Source: CAD feature listing. Evaluate the final solid. Frame: model axes, mm. Give positions to 0.01 mm unless a question says otherwise; leave off trailing zeros. Loops run counter-clockwise (first coordinate to the right, second up) from the corner with the lowest first, then second, coordinate; pieces in that order, holes last. Notation, with made-up numbers: (54, -30.75) -> (95, -30.75) arc R21 ccw to (95, 7.25) -> close; hole circle Ø7 at (-9.75, 35). An arc over 180 degrees is marked (long way). Put each result on its own line as item: value.
```python
from build123d import *

# Parameters (mm, degrees)
SKETCH_1_W         = 8
SKETCH_1_H         = 8
EXTRUDE_1_DEPTH    = 35
HOLE_WIZARD_M4_1_D = 3.3


with BuildPart() as part:
    # 草图1 → 凸台-拉伸1 (new body)
    with BuildSketch(Plane.XY):
        Rectangle(SKETCH_1_W, SKETCH_1_H)
    extrude(amount=EXTRUDE_1_DEPTH)

    # M4 螺纹孔1 (through all)
    with Locations(Plane(origin=(0, -4, 0), x_dir=(-1, 0, 0), z_dir=(0, -1, 0))):
        with Locations((0, -12), (0, -4)):
            Hole(HOLE_WIZARD_M4_1_D / 2)


solid = part.part
```
(1) Section A-A on y = 1.25. Return loops of the section in (x, z).
Calculated:
outline: (-4, 0) -> (4, 0) -> (4, 35) -> (-4, 35) -> close; hole circle Ø3.3 at (0, 4); hole circle Ø3.3 at (0, 12)
(2) Section C-C on z = 4. Return loops of the section in (x, y).
Calculated:
outline: (-4, -4) -> (-1.65, -4) -> (-1.65, 4) -> (-4, 4) -> close; (1.65, -4) -> (4, -4) -> (4, 4) -> (1.65, 4) -> close
(3) Draft query along X for faces 1 (the cylindrical face through (-0.4, 0.1, 13.6)), 2 (the flat face through (0, 4, 17)), 3 (the flat face through (4, 0, 17)). Return one class per face: released by +X, released by -X, zero draft, split by the parting line, or undercut.
Calculated:
face 1: undercut
face 2: zero draft
face 3: released by +X
(4) First-contact query: P1, Ø2.5, axis at x = 0, z = 4, coming from the +Y side. Flat tip, straight axial feed; report the tip coordinate or a pass-through.
Calculated:
P1: passes through
(5) Section B-B on x = 0. Return loops of the section in (y, z), then the cut area to 3 significant figures.
Calculated:
outline: (-4, 0) -> (4, 0) -> (4, 2.35) -> (-4, 2.35) -> close; (-4, 5.65) -> (4, 5.65) -> (4, 10.35) -> (-4, 10.35) -> close; (-4, 13.65) -> (4, 13.65) -> (4, 35) -> (-4, 35) -> close
area: 227 mm²
(6) Line query: probe 1 along Z at (x, y) = (0, 1.75); probe 2 along Z at (x, y) = (1.25, 3.75); probe 3 along X at (y, z) = (0.5, 4). Output: solid intervals per line, ascending. Write a range as from..to.
Calculated:
probe 1: z = 0..2.35, 5.65..10.35, 13.65..35
probe 2: z = 0..2.92, 5.08..10.92, 13.08..35
probe 3: x = -4..-1.65, 1.65..4
